from build123d import *

# Parameters (mm, degrees)
SKETCH_1_W                = 300
SKETCH_1_H                = 26
EXTRUDE_1_DEPTH           = 1
HOLE_WIZARD_5_0_5_1_D     = 5
HOLE_WIZARD_5_0_5_1_DEPTH = 5
HOLE_WIZARD_5_0_5_1_TIP   = 1.502151548


with BuildPart() as part:
    # 草图1 → 凸台-拉伸1 (new body)
    with BuildSketch(Plane.XY):
        with Locations((0, 13)):
            Rectangle(SKETCH_1_W, SKETCH_1_H)
    extrude(amount=EXTRUDE_1_DEPTH)

    # Ø5.0 (5) 直径孔1
    with Locations(Plane.XY.offset(1)):
        with Locations((-145, 13), (145, 13)):
            Hole(HOLE_WIZARD_5_0_5_1_D / 2, depth=HOLE_WIZARD_5_0_5_1_DEPTH)
            with Locations((0, 0, -(HOLE_WIZARD_5_0_5_1_DEPTH + HOLE_WIZARD_5_0_5_1_TIP / 2))):  # 118° drill point
                Cone(0, HOLE_WIZARD_5_0_5_1_D / 2, HOLE_WIZARD_5_0_5_1_TIP, mode=Mode.SUBTRACT)


solid = part.part
Geometry: final body of the model. Coordinates: model frame, mm. Round coordinates to 2 decimals unless told otherwise and drop trailing zeros. Order: outer loops, then holes, each group sorted by start corner. A loop starts at its lowest first (then second) coordinate and runs counter-clockwise, first axis right, second up. Notation, with made-up numbers: (-35, 70.25) - (-10, 70.25) arc R22 cw to (-10, 94.25) - close; hole circle Ø3 at (-10, 39). An arc over 180 degrees is marked (long way). Write each question's results on one line, items separated by ' | '.
Item 1: Section A-A, the plane y = 13. Return the cut outline in (x, z), and give its area (3 significant figures).
Completed:
outline: (-150, 0) - (-147.5, 0) - (-147.5, 1) - (-150, 1) - close; (-142.5, 0) - (142.5, 0) - (142.5, 1) - (-142.5, 1) - close; (147.5, 0) - (150, 0) - (150, 1) - (147.5, 1) - close | area: 290 mm^2
Item 2: Mould query, pull axis X, two halves, no side actions, for faces 1 (the flat face through (-2, 13, 1)), 2 (the cylindrical face through (-147.31, 12.04, 0.49)). Classes: pulls with the +X half, pulls with the -X half, needs draft (parallel to the pull), parting line crosses it, or undercut.
Completed:
face 1: needs draft | face 2: undercut
Item 3: Section B-B, the plane x = 145. Return the cut outline in (y, z).
Completed:
outline: (0, 0) - (10.5, 0) - (10.5, 1) - (0, 1) - close; (15.5, 0) - (26, 0) - (26, 1) - (15.5, 1) - close
Item 4: Material intervals for line 1 along X through (y, z) = (14.25, 0.3); line 2 along Y through (x, z) = (145, 0.45), sorted ascending. Write a range as [from, to].
Completed:
line 1: [-150, -147.17], [-142.83, 142.83], [147.17, 150] | line 2: [0, 10.5], [15.5, 26]
